from build123d import *

# Parameters (mm, degrees)
SKETCH_1_W          = 22
SKETCH_1_H          = 8
SKETCH_1_R          = 1.5
EXTRUDE_1_DEPTH     = 8
SKETCH_2_R          = 1.5
CUT_EXTRUDE_1_DEPTH = 16.779733838


with BuildPart() as part:
    # 草图1 → 凸台-拉伸1 (new body)
    with BuildSketch(Plane.XY):
        Rectangle(SKETCH_1_W, SKETCH_1_H)
        with Locations((-6, 0)):
            Circle(SKETCH_1_R, mode=Mode.SUBTRACT)
        with Locations((2, 0)):
            Circle(SKETCH_1_R, mode=Mode.SUBTRACT)
    extrude(amount=EXTRUDE_1_DEPTH)

    # 草图2 → 切除-拉伸1 (cut, through all)
    with BuildSketch(Plane(origin=(0, 4, 0), x_dir=(1, 0, 0), z_dir=(0, 1, 0))):
        with Locations(Location((6, -4, 0), (0, 0, 180))):
            Circle(SKETCH_2_R)
        with Locations(Location((-2, -4, 0), (0, 0, 180))):
            Circle(SKETCH_2_R)
    extrude(amount=-CUT_EXTRUDE_1_DEPTH, mode=Mode.SUBTRACT)


solid = part.part
Model file for the job. Use its own axes, mm. Give positions to 0.01 mm unless a question says otherwise; leave off trailing zeros. Order: outer loops, then holes, each group sorted by start corner. A loop starts at its lowest first (then second) coordinate and runs counter-clockwise, first axis right, second up. Notation, with made-up numbers: (41.5, -20.75) - (80.5, -20.75) arc R24 cw to (80.5, -0.75) - close; hole circle Ø3 at (-28.75, 37.5). An arc over 180 degrees is marked (long way). Return JSON: item names as keys, results as strings.
1) Cut at C-C, the plane y = -0.5. Give the cut face in (x, z), plus the area to 3 significant figures.
Geometry says:
{"outline": "(-11, 0) - (-7.41, 0) - (-7.41, 8) - (-11, 8) - close; (-4.59, 0) - (0.59, 0) - (0.59, 8) - (-4.59, 8) - close; (3.41, 0) - (11, 0) - (11, 8) - (3.41, 8) - close; hole circle Ø3 at (-2, 4); hole circle Ø3 at (6, 4)", "area": "117 mm²"}
2) Cut at A-A, the plane x = -2. Give the cut face in (y, z), plus the area to 3 significant figures.
Geometry says:
{"outline": "(-4, 0) - (4, 0) - (4, 2.5) - (-4, 2.5) - close; (-4, 5.5) - (4, 5.5) - (4, 8) - (-4, 8) - close", "area": "40.0 mm²"}
3) Cut at B-B, the plane z = 4.25. Give the cut face in (x, y).
Geometry says:
{"outline": "(-11, -4) - (-3.48, -4) - (-3.48, 4) - (-11, 4) - close; (-0.52, -4) - (4.52, -4) - (4.52, 4) - (-0.52, 4) - close; (7.48, -4) - (11, -4) - (11, 4) - (7.48, 4) - close; hole circle Ø3 at (-6, 0); hole circle Ø3 at (2, 0)"}
4) Pull direction Y, two halves, no side cores. Call faces 1 (the flat face through (0, -4, 4)), 2 (the cylindrical face through (-7.2, -0.9, 3.9)), 3 (the flat face through (-11, 0, 4)): pulls with the +Y half, pulls with the -Y half, needs draft (parallel to the pull), parting line crosses it, or undercut.
Geometry says:
{"face 1": "pulls with the -Y half", "face 2": "undercut", "face 3": "needs draft"}
5) Probe line 1 (Z direction, x = 6, y = -0.5); line 2 (X direction, y = 3.75, z = 5); line 3 (X direction, y = -1.25, z = 3.25). List the from-to ranges inside material, lowest first. Write a range as from..to.
Geometry says:
{"line 1": "0..2.5, 5.5..8", "line 2": "-11..-3.12, -0.88..4.88, 7.12..11", "line 3": "-11..-6.83, -5.17..-3.3, -0.7..1.17, 2.83..4.7, 7.3..11"}
6) Cut at D-D, the plane y = -3.25. Give the cut face in (x, z), plus the area to 3 significant figures.
Geometry says:
{"outline": "(-11, 0) - (11, 0) - (11, 8) - (-11, 8) - close; hole circle Ø3 at (-2, 4); hole circle Ø3 at (6, 4)", "area": "162 mm²"}
